Geometry check sheet. Reference: the model listing, model coordinates, mm. A direction names the side the tool comes from. Coordinates: 2 decimals unless noted, no trailing zeros. Write each loop counter-clockwise with the first axis right and the second up, starting at its lowest first coordinate (ties: lowest second). Pieces come first, ordered by that corner, then holes. Notation, with made-up numbers: (-18, 80) -> (29, 80) arc R19 cw to (29, 101) -> close; hole circle Ø7 at (64.25, 24). An arc over 180 degrees is marked (long way). Answer in a Markdown table with one row per item. Add a question column.
1. Set-up check for faces 1 (the cylindrical face through (5.894, 0.259, 17.944)), 2 (the flat face through (2, 6, 4)), 3 (the cylindrical face through (-7.493, 0.33, 0.986)): record each of +Z, -Z, +X, -X, +Y, -Y from which the full face is reachable in a straight line by a thin tool's end or side.
2. Cross-section at B-B on y = -6.5. Record the cut outline in (x, z), and give its area (3 significant figures).
3. Scan lines: L1, parallel to Y at x = 0, z = 2.5; L2, parallel to Y at x = 0, z = 16; L3, parallel to Z at x = 2, y = -5.75. Record each from-to range of solid material in increasing order. Write a range as from..to.
4. Cross-section at A-A on x = 0. Record the cut outline in (y, z).
5. Cross-section at D-D on z = 9.75. Record the cut outline in (x, y).
6. Mould release check, pull along X, two halves, no side actions. Record for faces 4 (the cylindrical face through (3, 0, 6)), 5 (the flat face through (6.896, -4.056, 16.93)), 6 (the flat face through (-6.961, -3.944, 16.93)): pulls with the +X half, pulls with the -X half, needs draft (parallel to the pull), parting line crosses it, or undercut.
7. Cross-section at C-C on z = 17.5. Record the cut outline in (x, y), and give its area (3 significant figures).
8. Depth check by flat-ended pin: P1, Ø5, axis at x = -2.5, z = 7.5, coming from the -Y side; P2, Ø1.5, axis at x = -7, y = 6.5, coming from the -Z side; P3, Ø6, axis at y = 3, z = 5, coming from the +X side. Enter the tip coordinate at first touch or a pass-through.
```python
from build123d import *

# Parameters (mm, degrees)
SKETCH1_R               = 7.5
BOSS_EXTRUDE1_DEPTH     = 2
SKETCH2_R               = 6
BOSS_EXTRUDE2_DEPTH     = 2
SKETCH3_R               = 7.5
BOSS_EXTRUDE3_DEPTH     = 8
BOSS_EXTRUDE4_DEPTH     = 10
SKETCH5_R               = 3
CUT_EXTRUDE1_DEPTH      = 26.166114784
G1_4_TAPPED_HOLE1_D     = 11.8
G1_4_TAPPED_HOLE1_DEPTH = 8
G1_4_TAPPED_HOLE1_TIP   = 3.545077652


with BuildPart() as part:
    # Sketch1 → Boss-Extrude1 (new body)
    with BuildSketch(Plane.XY):
        Circle(SKETCH1_R)
    extrude(amount=BOSS_EXTRUDE1_DEPTH)

    # Sketch2 → Boss-Extrude2 (add)
    with BuildSketch(Plane.XY.offset(2)):
        Circle(SKETCH2_R)
    extrude(amount=BOSS_EXTRUDE2_DEPTH)

    # Sketch3 → Boss-Extrude3 (add)
    with BuildSketch(Plane.XY.offset(4)):
        Circle(SKETCH3_R)
    extrude(amount=BOSS_EXTRUDE3_DEPTH)

    # Sketch4 → Boss-Extrude4 (add)
    with BuildSketch(Plane.XY.offset(12)):
        Polygon((9.237604307, 0), (4.618802154, 8), (-4.618802154, 8), (-9.237604307, 0), (-4.618802154, -8), (4.618802154, -8), align=None)
    extrude(amount=BOSS_EXTRUDE4_DEPTH)

    # Sketch5 → Cut-Extrude1 (cut, through all)
    with BuildSketch(Plane(origin=(0, 0, 0), x_dir=(-1, 0, 0), z_dir=(0, 0, -1))):
        Circle(SKETCH5_R)
    extrude(amount=-CUT_EXTRUDE1_DEPTH, mode=Mode.SUBTRACT)

    # G1/4 Tapped Hole1
    with Locations(Plane.XY.offset(22)):
        with Locations((0, 0)):
            Hole(G1_4_TAPPED_HOLE1_D / 2, depth=G1_4_TAPPED_HOLE1_DEPTH)
            with Locations((0, 0, -(G1_4_TAPPED_HOLE1_DEPTH + G1_4_TAPPED_HOLE1_TIP / 2))):  # 118° drill point
                Cone(0, G1_4_TAPPED_HOLE1_D / 2, G1_4_TAPPED_HOLE1_TIP, mode=Mode.SUBTRACT)


solid = part.part
```
Results found:
| question | item | result |
|---|---|---|
| 1 | face 1 | +Z |
| 1 | face 2 | none |
| 1 | face 3 | -Z |
| 2 | outline | (-5.48, 12) -> (-3.74, 12) -> (-3.74, 4) -> (3.74, 4) -> (3.74, 12) -> (5.48, 12) -> (5.48, 22) -> (-5.48, 22) -> close; (-3.74, 0) -> (3.74, 0) -> (3.74, 2) -> (-3.74, 2) -> close |
| 2 | area | 185 mm^2 |
| 3 | L1 | y = -6..-3, 3..6 |
| 3 | L2 | y = -8..-5.9, 5.9..8 |
| 3 | L3 | z = 0..2, 4..22 |
| 4 | outline | (-8, 12) -> (-7.5, 12) -> (-7.5, 4) -> (-6, 4) -> (-6, 2) -> (-7.5, 2) -> (-7.5, 0) -> (-3, 0) -> (-3, 12.26) -> (-5.9, 14) -> (-5.9, 22) -> (-8, 22) -> close; (3, 0) -> (7.5, 0) -> (7.5, 2) -> (6, 2) -> (6, 4) -> (7.5, 4) -> (7.5, 12) -> (8, 12) -> (8, 22) -> (5.9, 22) -> (5.9, 14) -> (3, 12.26) -> close |
| 5 | outline | circle Ø15 at (0, 0); hole circle Ø6 at (0, 0) |
| 6 | face 4 | undercut |
| 6 | face 5 | pulls with the +X half |
| 6 | face 6 | pulls with the -X half |
| 7 | outline | (-9.24, 0) -> (-4.62, -8) -> (4.62, -8) -> (9.24, 0) -> (4.62, 8) -> (-4.62, 8) -> close; hole circle Ø11.8 at (0, 0) |
| 7 | area | 112 mm^2 |
| 8 | P1 | stops at y = -7.5 |
| 8 | P2 | passes through |
| 8 | P3 | stops at x = 7.5 |
